Check sheet for the modelled part. Datum: model origin and axes. Units: mm. Face numbers are marked on the shaded views. A direction names the side the tool comes from. Round coordinates to 2 decimals unless told otherwise and drop trailing zeros. Order: outer loops, then holes, each group sorted by start corner. A loop starts at its lowest first (then second) coordinate and runs counter-clockwise, first axis right, second up.
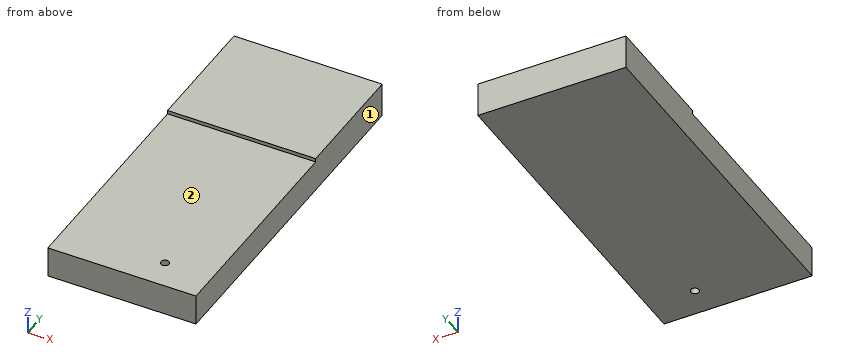
```python
from build123d import *

# Parameters (mm, degrees)
SKETCH_1_W          = 60
SKETCH_1_H          = 140
EXTRUDE_1_DEPTH     = 14
SKETCH_2_W          = 60
SKETCH_2_H          = 90
CUT_EXTRUDE_1_DEPTH = 1.5
HOLE_WIZARD_M4_1_D  = 3.3


with BuildPart() as part:
    # 草图1 → 凸台-拉伸1 (new body)
    with BuildSketch(Plane.XY):
        Rectangle(SKETCH_1_W, SKETCH_1_H)
    extrude(amount=EXTRUDE_1_DEPTH)

    # 草图2 → 切除-拉伸1 (cut)
    with BuildSketch(Plane.XY.offset(14)):
        with Locations((0, -25)):
            Rectangle(SKETCH_2_W, SKETCH_2_H)
    extrude(amount=-CUT_EXTRUDE_1_DEPTH, mode=Mode.SUBTRACT)

    # M4 螺纹孔1 (through all)
    with Locations(Plane(origin=(0, 0, 0), x_dir=(-1, 0, 0), z_dir=(0, 0, -1))):
        with Locations((-11, -58)):
            Hole(HOLE_WIZARD_M4_1_D / 2)


solid = part.part
```
Item 1: Scan lines: line 1 along Y through (x, z) = (11, 5.25); line 2 along Z through (x, y) = (15, -1); line 3 along Y through (x, z) = (6, 13). Record each from-to range of solid material in increasing order.
Answer:
line 1: y = -70 to -59.65, -56.35 to 70
line 2: z = 0 to 12.5
line 3: y = 20 to 70
Item 2: Sectioned sample at A-A (y = -58). Record the cut outline in (x, z).
Answer:
outline: (-30, 0) - (9.35, 0) - (9.35, 12.5) - (-30, 12.5) - close; (12.65, 0) - (30, 0) - (30, 12.5) - (12.65, 12.5) - close
Item 3: Access from +Z, -Z, +X, -X, +Y, -Y to the whole of each face (thin tool, end or side, straight path). Record for the marked faces 1 and 2.
Answer:
face 1: +Z, -Z, +X, +Y, -Y
face 2: +Z, +X, -X, -Y
Item 4: Sectioned sample at C-C (y = -22.5). Record the cut outline in (x, z).
Answer:
outline: (-30, 0) - (30, 0) - (30, 12.5) - (-30, 12.5) - close
Item 5: Sectioned sample at B-B (x = 11). Record the cut outline in (y, z).
Answer:
outline: (-70, 0) - (-59.65, 0) - (-59.65, 12.5) - (-70, 12.5) - close; (-56.35, 0) - (70, 0) - (70, 14) - (20, 14) - (20, 12.5) - (-56.35, 12.5) - close
Item 6: Go/stop test with flat-tipped pins: P1, Ø12, axis at x = -21, y = -1, coming from the -Z side; P2, Ø8, axis at x = -12.5, y = -33, coming from the +Z side; P3, Ø1.2, axis at x = 5.5, z = 13.5, coming from the -Y side. Record where each tip stops, or that it passes through.
Answer:
P1: stops at z = 0
P2: stops at z = 12.5
P3: stops at y = 20
